For this review, take the finished solid that the model builds, in its own axes (mm). A direction names the side the tool comes from. Give positions to 0.01 mm unless a question says otherwise; leave off trailing zeros. Loops run counter-clockwise (first coordinate to the right, second up) from the corner with the lowest first, then second, coordinate; pieces in that order, holes last.
```python
from build123d import *

# Parameters (mm, degrees)
EXTRUDE_1_DEPTH    = 50
SKETCH_3_W         = 8
SKETCH_3_H         = 5
EXTRUDE_2_DEPTH    = 50
CHAMFER_1_SIZE     = 1
CHAMFER_2_SIZE     = 1
CHAMFER_3_SIZE     = 3
HOLE_WIZARD_M3_1_D = 3.4
CHAMFER_4_SIZE     = 2


with BuildPart() as part:
    # 草图1 → 凸台-拉伸1 (new body)
    with BuildSketch(Plane.XY):
        Polygon((15, 0), (-15, 0), (-15, 15), (-6.25, 15), (-6.25, 10), (-10, 10), (-10, 5), (10, 5), (10, 10), (6.25, 10), (6.25, 15), (15, 15), align=None)
    extrude(amount=EXTRUDE_1_DEPTH)

    # 草图3 → 凸台-拉伸2 (add)
    with BuildSketch(Plane.XY.offset(50)):
        with Locations((-19, 2.5)):
            Rectangle(SKETCH_3_W, SKETCH_3_H)
        with Locations((19, 2.5)):
            Rectangle(SKETCH_3_W, SKETCH_3_H)
    extrude(amount=-EXTRUDE_2_DEPTH)

    # 倒角1
    chamfer_1_edges = [part.edges().sort_by_distance(p)[0] for p in [
        (8.125, 10, 50),
        (10, 7.5, 50),
        (0, 5, 50),
        (-10, 7.5, 50),
        (-8.125, 10, 50),
    ]]
    chamfer(chamfer_1_edges, length=CHAMFER_1_SIZE)

    # 倒角2
    chamfer_2_edges = [part.edges().sort_by_distance(p)[0] for p in [
        (-8.125, 10, 0),
        (-10, 7.5, 0),
        (0, 5, 0),
        (10, 7.5, 0),
        (8.125, 10, 0),
    ]]
    chamfer(chamfer_2_edges, length=CHAMFER_2_SIZE)

    # 倒角3
    chamfer_3_edges = [part.edges().sort_by_distance(p)[0] for p in [
        (-23, 2.5, 50),
        (-23, 2.5, 0),
        (23, 2.5, 50),
        (23, 2.5, 0),
    ]]
    chamfer(chamfer_3_edges, length=CHAMFER_3_SIZE)

    # M3 间隙孔1 (through all)
    with Locations(Plane(origin=(0, 5, 0), x_dir=(1, 0, 0), z_dir=(0, 1, 0))):
        with Locations((-19.5, -10), (-19.5, -40), (19.5, -40), (19.5, -10)):
            Hole(HOLE_WIZARD_M3_1_D / 2)

    # 倒角4
    chamfer_4_edges = [part.edges().sort_by_distance(p)[0] for p in [
        (-15, 15, 25),
        (15, 15, 25),
    ]]
    chamfer(chamfer_4_edges, length=CHAMFER_4_SIZE)


solid = part.part
```
Item 1: The part is to be moulded in two halves that separate along Y. For faces 1 (the flat face through (8, 10, 25)), 2 (the flat face through (-22, 2, 48)), 3 (the flat face through (-8, 10, 25)), 4 (the flat face through (19, 5, 25)), say which applies: released by +Y, released by -Y, zero draft, split by the parting line, or undercut.
Answer:
face 1: undercut
face 2: zero draft
face 3: undercut
face 4: released by +Y
Item 2: For L1, parallel to Z at x = -19.5, y = 2.35; L2, parallel to X at y = 1.9, z = 10; L3, parallel to Y at x = 7.5, z = 14.5, list the stretches that pass through material, from the lowest coordinate up.
Answer:
L1: z = 0 to 8.3, 11.7 to 38.3, 41.7 to 50
L2: x = -23 to -21.2, -17.8 to 17.8, 21.2 to 23
L3: y = 0 to 5, 10 to 15
Item 3: Clearance check with flat-ended pins moving along their axes: pin 1 Ø1.5 at (y, z) = (6.5, 14) entering from -X; pin 2 Ø1.5 at (y, z) = (7, 28.5) entering from +X; pin 3 Ø4 at (x, z) = (19.5, 10) entering from +Y. State where each tip first meets the part, or that it passes through.
Answer:
pin 1: stops at x = -15
pin 2: stops at x = 15
pin 3: stops at y = 5
Item 4: Take a section at C-C on z = 16.5. Give the boundary of the cut face in (x, y).
Answer:
outline: (-23, 0) - (23, 0) - (23, 5) - (15, 5) - (15, 13) - (13, 15) - (6.25, 15) - (6.25, 10) - (10, 10) - (10, 5) - (-10, 5) - (-10, 10) - (-6.25, 10) - (-6.25, 15) - (-13, 15) - (-15, 13) - (-15, 5) - (-23, 5) - close
Item 5: Take a section at A-A on z = 40. Give the boundary of the cut face in (x, y), and give its area (4 significant figures).
Answer:
outline: (-23, 0) - (-21.2, 0) - (-21.2, 5) - (-23, 5) - close; (-17.8, 0) - (17.8, 0) - (17.8, 5) - (15, 5) - (15, 13) - (13, 15) - (6.25, 15) - (6.25, 10) - (10, 10) - (10, 5) - (-10, 5) - (-10, 10) - (-6.25, 10) - (-6.25, 15) - (-13, 15) - (-15, 13) - (-15, 5) - (-17.8, 5) - close; (21.2, 0) - (23, 0) - (23, 5) - (21.2, 5) - close
area: 329.5 mm2
Item 6: Take a section at D-D on x = -4.5. Give the boundary of the cut face in (y, z), and give its area (3 significant figures).
Answer:
outline: (0, 0) - (4, 0) - (5, 1) - (5, 49) - (4, 50) - (0, 50) - close
area: 249 mm2
Item 7: Tool access review of faces 5 (the flat face through (-6.25, 13, 25)), 6 (the flat face through (-19, 5, 25)), 7 (the flat face through (15, 9, 25)): name each direction out of +Z, -Z, +X, -X, +Y, -Y from which nothing blocks a thin tool from reaching the whole face with its end or side.
Answer:
face 5: +Z, -Z, +Y
face 6: +Z, -Z, -X, +Y
face 7: +Z, -Z, +X, +Y
Item 8: Take a section at B-B on y = 9. Give the boundary of the cut face in (x, z), and give its area (3 significant figures).
Answer:
outline: (-15, 0) - (-11, 0) - (-10, 1) - (-10, 49) - (-11, 50) - (-15, 50) - close; (10, 1) - (11, 0) - (15, 0) - (15, 50) - (11, 50) - (10, 49) - close
area: 498 mm2
